Verification items for the finished model (mm, model axes). A direction names the side the tool comes from. Coordinates: 2 decimals unless noted, no trailing zeros. Loops run counter-clockwise (first coordinate to the right, second up) from the corner with the lowest first, then second, coordinate; pieces in that order, holes last.
Q1. Sectioned sample at D-D (y = -39). Enter the section's corners in (x, z), then the cut area to 3 significant figures.
Q2. Sectioned sample at A-A (z = 0). Enter the section's corners in (x, y), then the cut area to 3 significant figures.
Q3. Sectioned sample at B-B (x = 0). Enter the section's corners in (y, z), then the cut area to 3 significant figures.
Q4. Material ranges on probe 1 along Z at (x, y) = (7, 62.5); probe 2 along X at (y, z) = (13.5, 0), recorded low to high.
Q5. Go/stop test with flat-tipped pins: P1, Ø1.5, axis at y = 23, z = 2, coming from the +X side; P2, Ø4.5, axis at y = 80, z = 2.5, coming from the +X side; P3, Ø0.8, axis at x = 3, z = 11, coming from the +Y side; P4, Ø1.5, axis at y = 52, z = -15, coming from the +X side. Record where each tip stops, or that it passes through.
Q6. Access from +Z, -Z, +X, -X, +Y, -Y to the whole of each face (thin tool, end or side, straight path). Record for faces 1 (the face through (0, 75, 10)), 2 (the face through (-10, 75, 0)), 3 (the face through (0, 75, -10)), 4 (the face through (0, 90.3, 0)), 5 (the face through (11, 59.3, 0)).
Q7. Sectioned sample at C-C (y = 13). Enter the section's corners in (x, z), then the cut area to 3 significant figures.
```python
from build123d import *

# Parameters (mm, degrees)
STEM_SHAFT_SKETCH_25_4_R     = 12.7
STEM_SHAFT_25_4_DEPTH        = 90.3
DRIVE_START                  = -31
DRIVE_SQUARE_FLATS_CUT_DEPTH = 31
STEM_START                   = 31
STEM_BOSS_SKETCH_R           = 12.7
STEM_BOSS_31MM_DEPTH         = 31


with BuildPart() as part:
    # Stem Shaft Sketch _25.4 → Stem Shaft _25.4 (new body)
    with BuildSketch(Plane(origin=(0, 0, 0), x_dir=(1, 0, 0), z_dir=(0, 1, 0))):
        with Locations(Location((0, 0, 0), (0, 0, 270))):
            Circle(STEM_SHAFT_SKETCH_25_4_R)
    extrude(amount=STEM_SHAFT_25_4_DEPTH)

    # Drive Square Flats Sketch → Drive Square Flats Cut (cut)
    with BuildSketch(Plane(origin=(0, 90.3, 0), x_dir=(1, 0, 0), z_dir=(0, 1, 0)).offset(DRIVE_START)):
        with BuildLine():
            ThreePointArc((-7.82879301, -10), (0, -12.7), (7.82879301, -10))
            Line((7.82879301, -10), (-7.82879301, -10))
        make_face()
        with BuildLine():
            Line((-10, -7.82879301), (-10, 7.82879301))
            ThreePointArc((-10, 7.82879301), (-12.7, 0), (-10, -7.82879301))
        make_face()
        with BuildLine():
            Line((-7.82879301, 10), (7.82879301, 10))
            ThreePointArc((7.82879301, 10), (0, 12.7), (-7.82879301, 10))
        make_face()
        with BuildLine():
            Line((10, 7.82879301), (10, 0))
            Line((10, 0), (10, -7.82879301))
            ThreePointArc((10, -7.82879301), (12.006040147, -4.140652123), (12.7, 0))
            ThreePointArc((12.7, 0), (12.006040147, 4.140652123), (10, 7.82879301))
        make_face()
    extrude(amount=DRIVE_SQUARE_FLATS_CUT_DEPTH, mode=Mode.SUBTRACT)

    # Stem Boss Sketch → Stem Boss 31mm (add)
    with BuildSketch(Plane.XZ.offset(STEM_START)):
        with Locations(Location((0, 0, 0), (0, 0, 270))):
            Circle(STEM_BOSS_SKETCH_R)
    extrude(amount=-STEM_BOSS_31MM_DEPTH)


with BuildPart() as body_2:
    # Ball Profile Sketch → Valve Ball (revolve)
    with BuildSketch(Plane.XY):
        with BuildLine():
            Line((-25.3, -30.67), (25.3, -30.67))
            ThreePointArc((25.3, -30.67), (0, -55.97), (-25.3, -30.67))
        make_face()
    revolve(axis=Axis((-25.3, -30.67, 0), (1, 0, 0)))

    # Combine1: union part
    add(part.part)


solid = body_2.part
```
Geometry check:
1. outline: circle Ø47.78 at (0, 0)
1. area: 1,790 mm2
2. outline: (-12.7, -8.79) arc R25.3 ccw (long way) to (12.7, -8.79) - (12.7, 59.3) - (10, 59.3) - (10, 90.3) - (-10, 90.3) - (-10, 59.3) - (-12.7, 59.3) - close
2. area: 4,300 mm2
3. outline: (-8.79, -12.7) - (59.3, -12.7) - (59.3, -10) - (90.3, -10) - (90.3, 10) - (59.3, 10) - (59.3, 12.7) - (-8.79, 12.7) arc R25.3 ccw (long way) to start
3. area: 4,300 mm2
4. probe 1: z = -10 to 10
4. probe 2: x = -12.7 to 12.7
5. P1: stops at x = 12.64
5. P2: stops at x = 10
5. P3: stops at y = 59.3
5. P4: passes through
6. face 1: +Z, +X, -X, +Y
6. face 2: +Z, -Z, -X, +Y
6. face 3: -Z, +X, -X, +Y
6. face 4: +Z, -Z, +X, -X, +Y
6. face 5: +Z, -Z, +X, +Y
7. outline: circle Ø25.4 at (0, 0)
7. area: 507 mm2
